Check sheet for the drawn part. Datum: minimum x, y, z corner. Units: mm. A direction names the side the tool comes from. Coordinates: 2 decimals unless noted, no trailing zeros. Write each loop counter-clockwise with the first axis right and the second up, starting at its lowest first coordinate (ties: lowest second). Pieces come first, ordered by that corner, then holes. Notation, with made-up numbers: (-4.5, 77.25) -> (48.5, 77.25) arc R12 cw to (48.5, 88.25) -> close; hole circle Ø4 at (-22.75, 37). An arc over 180 degrees is marked (long way). Write item = value, one per line. Start each with the question number.
(1) Section check B-B (z = 34). Record the cut outline in (x, y), plus the area to 3 significant figures.
(2) Section check A-A (x = 20). Record the cut outline in (y, z), plus the area to 3 significant figures.
(3) Set-up check for the marked faces 4, 5 and 6: record each of +Z, -Z, +X, -X, +Y, -Y from which the full face is reachable in a straight line by a thin tool's end or side.
(4) Material ranges on probe 1 along Y at (x, z) = (53, 22); probe 2 along X at (y, z) = (3.5, 36); probe 3 along Y at (x, z) = (54.5, 23.5), recorded low to high. Write a range as [from, to].
(5) Mould release check, pull along X, two halves, no side actions. Record for the marked faces 1, 2 and 3: released by +X, released by -X, zero draft, split by the parting line, or undercut.
(6) Section check C-C (y = 39). Record the cut outline in (x, z).
(7) Gauge pin test, flat ends, axial feed: pin 1 Ø23.5 at (y, z) = (32.5, 34) entering from -X; pin 2 Ø10 at (x, y) = (31, 49.5) entering from -Z; pin 3 Ø3 at (x, y) = (10.5, 24.5) entering from +Z; pin 4 Ø3 at (x, y) = (34, 52.5) entering from -Z. Record the tip position at first contact, or that the pin passes through.
(8) Section check D-D (y = 32.5). Record the cut outline in (x, z).
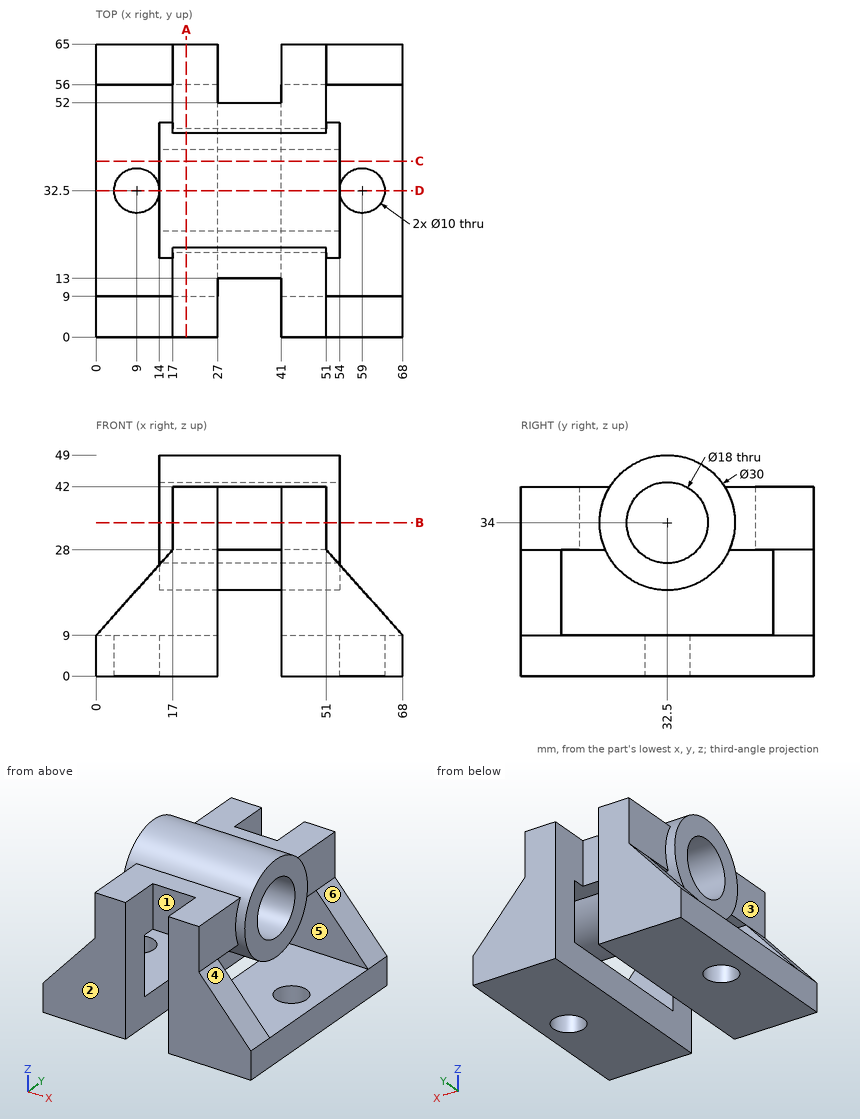
Response:
q1.outline = (14, 17.5) -> (17, 17.5) -> (17, 0) -> (27, 0) -> (27, 13) -> (41, 13) -> (41, 0) -> (51, 0) -> (51, 17.5) -> (54, 17.5) -> (54, 23.5) -> (14, 23.5) -> close; (14, 41.5) -> (54, 41.5) -> (54, 47.5) -> (51, 47.5) -> (51, 65) -> (41, 65) -> (41, 52) -> (27, 52) -> (27, 65) -> (17, 65) -> (17, 47.5) -> (14, 47.5) -> close
q1.area = 1,310 mm2
q2.outline = (0, 0) -> (65, 0) -> (65, 42) -> (45.19, 42) arc R15 ccw to (19.81, 42) -> (0, 42) -> close; hole (9, 9) -> (56, 9) -> (56, 28) -> (46.25, 28) arc R15 cw to (18.75, 28) -> (9, 28) -> close; hole circle Ø18 at (32.5, 34)
q2.area = 1,890 mm2
q3.face_4 = +Z, +X, -Y
q3.face_5 = +X, -X
q3.face_6 = +Z, +X, +Y
q4.probe_1 = [0, 9], [23.5, 41.5], [56, 65]
q4.probe_2 = [17, 27], [41, 51]
q4.probe_3 = [0, 9], [56, 65]
q5.face_1 = undercut
q5.face_2 = zero draft
q5.face_3 = released by -X
q6.outline = (0, 0) -> (27, 0) -> (27, 9) -> (0, 9) -> close; (14, 20.48) -> (54, 20.48) -> (54, 27.78) -> (14, 27.78) -> close; (14, 40.22) -> (54, 40.22) -> (54, 47.52) -> (14, 47.52) -> close; (41, 0) -> (68, 0) -> (68, 9) -> (41, 9) -> close
q7.pin_1 = 14
q7.pin_2 = 0
q7.pin_3 = 9
q7.pin_4 = 28
q8.outline = (0, 0) -> (4, 0) -> (4, 9) -> (0, 9) -> close; (14, 0) -> (27, 0) -> (27, 9) -> (14, 9) -> close; (14, 19) -> (54, 19) -> (54, 25) -> (14, 25) -> close; (14, 43) -> (54, 43) -> (54, 49) -> (14, 49) -> close; (41, 0) -> (54, 0) -> (54, 9) -> (41, 9) -> close; (64, 0) -> (68, 0) -> (68, 9) -> (64, 9) -> close
